```python
from build123d import *

# Parameters (mm, degrees)
CHAMFER1_SIZE = 1


with BuildPart() as part:
    # Sketch1 → Revolve2 (revolve)
    with BuildSketch(Plane.XY, mode=Mode.PRIVATE) as revolve2_sk:
        with BuildLine():
            Line((0, 0), (-10, 0))
            Line((-10, 0), (-15, 0))
            Line((-15, 0), (-430, 0))
            ThreePointArc((-430, 0), (-427.363961031, 6.363961031), (-421, 9))
            Line((-421, 9), (-15, 9))
            Line((-15, 9), (-15, 4.7))
            Line((-15, 4.7), (-10, 4.7))
            Line((-10, 4.7), (-10, 6))
            Line((-10, 6), (0, 6))
            Line((0, 6), (0, 0))
        make_face()
    revolve(revolve2_sk.sketch.rotate(Axis((-15, 0, 0), (-1, 0, 0)), 90), axis=Axis((-15, 0, 0), (-1, 0, 0)))

    # Chamfer1
    chamfer1_edges = [part.edges().sort_by_distance(p)[0] for p in [
        (0, 0, 6),
    ]]
    chamfer(chamfer1_edges, length=CHAMFER1_SIZE)


solid = part.part
```
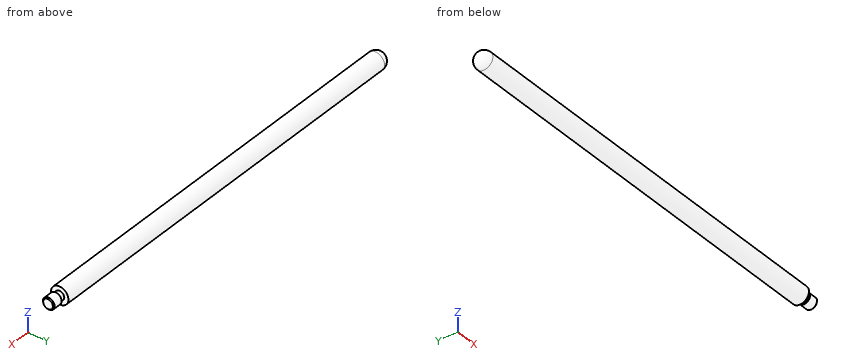
Could you check a few things on this model? Use its own coordinates, in mm. Round coordinates to 2 decimals unless told otherwise and drop trailing zeros. Loops run counter-clockwise (first coordinate to the right, second up) from the corner with the lowest first, then second, coordinate; pieces in that order, holes last.
Q1. Please list where these lines run through material, in increasing order: L1, parallel to Z at x = -258.5, y = 0.5; L2, parallel to X at y = -2.5, z = 4.25.
Q2. I want a section at A-A (z = 0). Write out the boundary of the cut face in (x, y), and give its area (3 significant figures).
Q3. For P1, Ø10, axis at y = -0.5, z = -6.5, coming from the -X side; P2, Ø1, axis at x = -188, y = 7, coming from the -Z side; P3, Ø4, axis at x = -282, z = -6.5, coming from the +Y side, each with a flat end and sliding along its axis, tell me the tip position at first contact or that it passes through.
Q4. I want a section at C-C (x = -210). Write out the boundary of the cut face in (y, z), and give its area (3 significant figures).
Answer below:
1. L1: z = -8.99 to 8.99
1. L2: x = -428.53 to -15, -10 to 0
2. outline: (-421, -9) - (-15, -9) - (-15, -4.7) - (-10, -4.7) - (-10, -6) - (-1, -6) - (0, -5) - (0, 5) - (-1, 6) - (-10, 6) - (-10, 4.7) - (-15, 4.7) - (-15, 9) - (-421, 9) arc R9 ccw to start
2. area: 7,600 mm2
3. P1: stops at x = -429.87
3. P2: stops at z = -6.22
3. P3: stops at y = 7.79
4. outline: circle Ø18 at (0, 0)
4. area: 254 mm2
